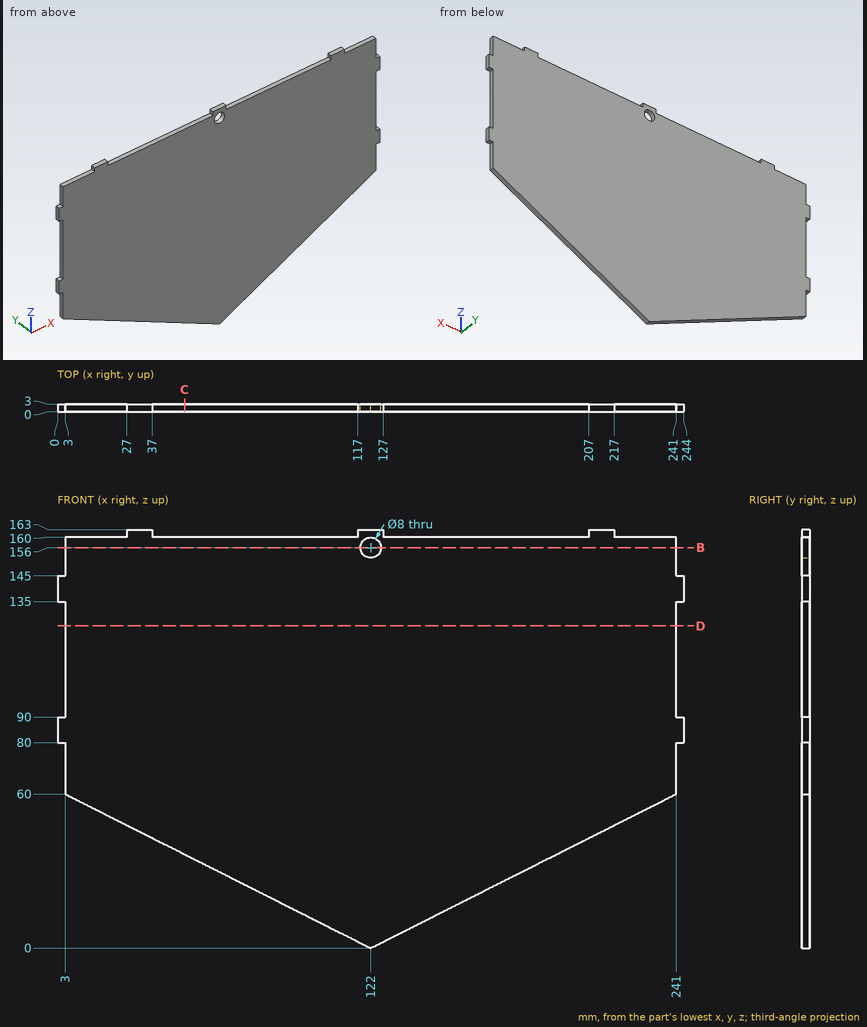
Study the drawing (mm; zero at the part's minimum x, y, z) and answer. Coordinates: 2 decimals unless noted, no trailing zeros. Write each loop counter-clockwise with the first axis right and the second up, starting at its lowest first coordinate (ties: lowest second). Pieces come first, ordered by that corner, then holes. Notation, with made-up numbers: (14, -3.75) - (40, -3.75) arc R10 ccw to (40, 10.25) - close; hole circle Ø1 at (46.5, -18.75). An arc over 180 degrees is marked (long way). Answer as a JSON object with one key per item and string values.
Q1. Given pin 1 Ø1.5 at (y, z) = (1, 153.5) entering from +X; pin 2 Ø0.9 at (x, y) = (161, 1.5) entering from +Z; pin 3 Ø1.5 at (x, y) = (243, 1.5) entering from +Z; pin 4 Ø10.5 at (x, z) = (122, 156) entering from +Y, each flat-ended and moving along its own axis, determine where each tip first touches the part or whether it passes through.
Results list:
{"pin 1": "stops at x = 241", "pin 2": "stops at z = 160", "pin 3": "stops at z = 145", "pin 4": "stops at y = 3"}
Q2. Find section B-B (z = 156). Write down the section's boundary in (x, y).
Results list:
{"outline": "(3, 0) - (118, 0) - (118, 3) - (3, 3) - close; (126, 0) - (241, 0) - (241, 3) - (126, 3) - close"}
Q3. Find section D-D (z = 125.5). Write down the section's boundary in (x, y).
Results list:
{"outline": "(3, 0) - (241, 0) - (241, 3) - (3, 3) - close"}
Q4. Consider L1, parallel to X at y = 2.05, z = 156; L2, parallel to X at y = 2.25, z = 115.5; L3, parallel to Z at x = 100, y = 0.55. Determine where each line is inside the solid, lowest interval first. Write a range as from..to.
Results list:
{"L1": "x = 3..118, 126..241", "L2": "x = 3..241", "L3": "z = 11.09..160"}
Q5. Find section C-C (x = 49.5). Write down the section's boundary in (y, z).
Results list:
{"outline": "(0, 36.55) - (3, 36.55) - (3, 160) - (0, 160) - close"}
